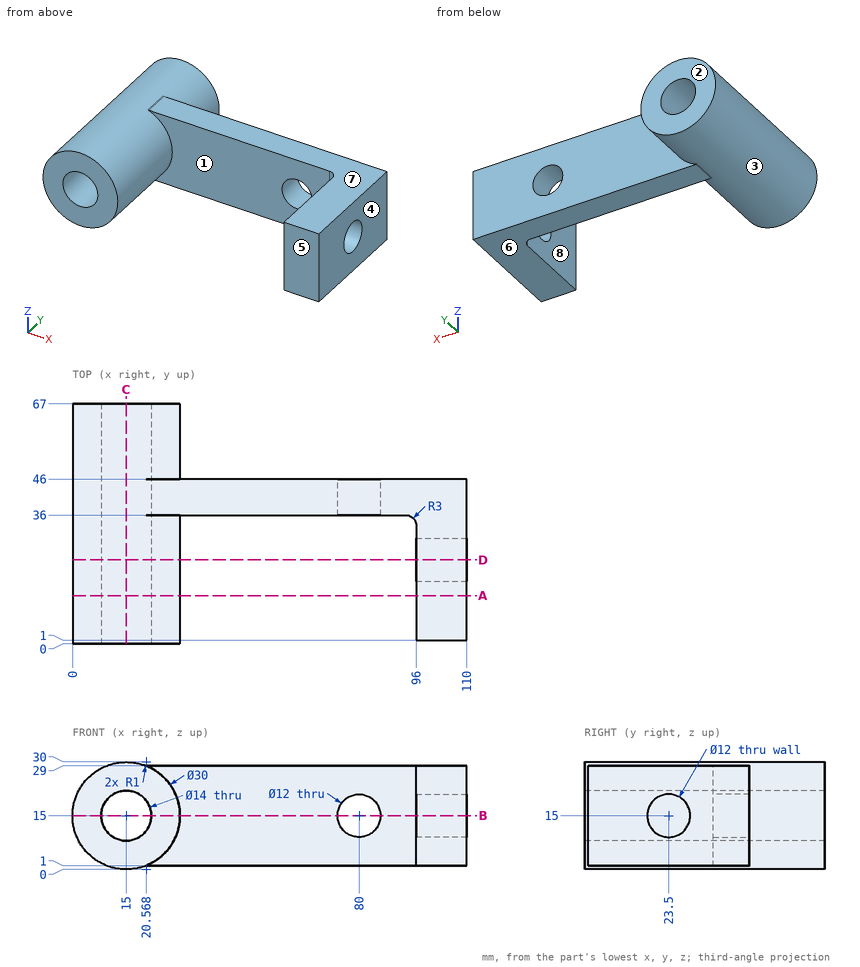
Study the drawing (mm; zero at the part's minimum x, y, z) and answer. A direction names the side the tool comes from. Coordinates: 2 decimals unless noted, no trailing zeros. Write each loop counter-clockwise with the first axis right and the second up, starting at its lowest first coordinate (ties: lowest second). Pieces come first, ordered by that corner, then holes. Notation, with made-up numbers: (56.25, -38.75) - (84.25, -38.75) arc R28 cw to (84.25, -18.75) - close; hole circle Ø8 at (13, 45.25). An arc over 180 degrees is marked (long way). Return JSON: item names as keys, results as strings. Group by question number.
1. Straight lines are drawn through the part: L1, parallel to X at y = 43, z = 15; L2, parallel to Y at x = 103.5, z = 15; L3, parallel to X at y = 8, z = 21 (1 decimal). For each, find the intervals that lie inside material, in ascending order.
2. A cutting plane is placed at B-B, the plane z = 15. Determine the outline of the cut face in (x, y).
3. Determine the mould class of the marked faces 1, 2, 3 and 4 for opening direction X: released by +X, released by -X, zero draft, split by the parting line, or undercut.
4. A cutting plane is placed at C-C, the plane x = 15. Determine the outline of the cut face in (y, z).
5. Which of the six approach directions +Z, -Z, +X, -X, +Y, -Y give full straight-line access (tool end or side, diameter ignored) to the marked faces 5, 6, 7 and 8?
6. A cutting plane is placed at D-D, the plane y = 23.5. Determine the outline of the cut face in (x, z), plus the area to 3 significant figures.
7. A cutting plane is placed at A-A, the plane y = 13.5. Determine the outline of the cut face in (x, z).
8. Given pin 1 (4 mm diameter, centred on x = 65, y = 46, fed in from +Z); pin 2 (1.5 mm diameter, centred on x = 18, y = 57, fed in from +Z); pin 3 (2 mm diameter, centred on y = 9, z = 22.5, fed in from -X); pin 4 (22.5 mm diameter, centred on x = 47.5, y = 14, fed in from +Z), each flat-ended and moving along its own axis, determine where each tip first touches the part or whether it passes through.
Ans:
{
 "1": {"L1": "0 to 8, 22 to 74, 86 to 110", "L2": "1 to 17.5, 29.5 to 46", "L3": "1.3 to 11.4, 18.6 to 28.7, 96 to 110"},
 "2": {"outline": "(0, 0) - (8, 0) - (8, 67) - (0, 67) - close; (22, 0) - (30, 0) - (30, 36) - (74, 36) - (74, 46) - (30, 46) - (30, 67) - (22, 67) - close; (86, 36) - (93, 36) arc R3 cw to (96, 33) - (96, 29.5) - (110, 29.5) - (110, 46) - (86, 46) - close; (96, 1) - (110, 1) - (110, 17.5) - (96, 17.5) - close"},
 "3": {"face 1": "undercut", "face 2": "zero draft", "face 3": "undercut", "face 4": "released by +X"},
 "4": {"outline": "(0, 0) - (67, 0) - (67, 8) - (0, 8) - close; (0, 22) - (67, 22) - (67, 30) - (0, 30) - close"},
 "5": {"face 5": "+Z, -Z, +X, -Y", "face 6": "-Z, +X, +Y, -Y", "face 7": "+Z, +X, +Y, -Y", "face 8": "+Z, -Z, -Y"},
 "6": {"outline": "circle Ø30 at (15, 15); (96, 1) - (110, 1) - (110, 9) - (96, 9) - close; (96, 21) - (110, 21) - (110, 29) - (96, 29) - close; hole circle Ø14 at (15, 15)", "area": "777 mm²"},
 "7": {"outline": "circle Ø30 at (15, 15); (96, 1) - (110, 1) - (110, 29) - (96, 29) - close; hole circle Ø14 at (15, 15)"},
 "8": {"pin 1": "z = 29", "pin 2": "z = 29.83", "pin 3": "x = 1.48", "pin 4": "through"}
}
